Here's how the part is built. I have some questions about the finished solid (model axes, mm). Coordinates: 2 decimals unless noted, no trailing zeros. Write each loop counter-clockwise with the first axis right and the second up, starting at its lowest first coordinate (ties: lowest second). Pieces come first, ordered by that corner, then holes.
Item 1: I'm going to push flat-ended pins straight in: P1, Ø3, axis at x = 7, y = -54.5, coming from the -Z side; P2, Ø7, axis at x = 0, y = -31, coming from the +Z side. Where does each tip first touch, or does it pass through?
Item 2: I want a section at D-D (z = 3.5). Count the separate pieces of the cut face and the enclosed holes in it, and give its area (3 significant figures).
Item 3: I want a section at B-B (y = 46). Please give me the cut outline in (x, z).
Item 4: Please list where these lines run through material, in increasing order: line 1 (Y direction, x = 0, z = 2.8); line 2 (Y direction, x = -20, z = -1.75); line 3 (Y direction, x = -22, z = -1).
Item 5: I want a section at C-C (x = 0). Please give me the cut outline in (y, z), and give its area (3 significant figures).
Item 6: I want a section at A-A (y = -54). Please give me the cut outline in (x, z).
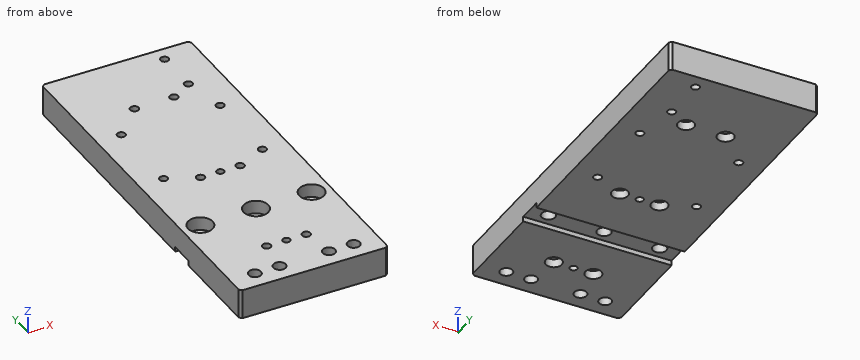
from build123d import *

# Parameters (mm, degrees)
SKETCH1_W                                           = 60
SKETCH1_H                                           = 150
BOSS_EXTRUDE1_DEPTH                                 = 6
M4_TAPPED_HOLE1_D                                   = 3.3
M4_TAPPED_HOLE2_D                                   = 3.3
M4_TAPPED_HOLE2_DEPTH                               = 15.5
M4_TAPPED_HOLE2_TIP                                 = 0.991420021
M6_TAPPED_HOLE2_D                                   = 5
BLIND_PIN_HOLE2_SIZE_MM_D                           = 5
CHAMFER1_SIZE                                       = 1
CBORE_FOR_M3_HEX_SOCKET_HEAD_CAP_SCREW1_D           = 3.4
CBORE_FOR_M3_HEX_SOCKET_HEAD_CAP_SCREW1_CBORE_D     = 6.5
CBORE_FOR_M3_HEX_SOCKET_HEAD_CAP_SCREW1_CBORE_DEPTH = 3.4
LPATTERN1_COUNT                                     = 3
LPATTERN1_PITCH                                     = 50
SKETCH20_R                                          = 1.5
CUT_EXTRUDE1_DEPTH                                  = 82.663945533
SKETCH21_W                                          = 60
SKETCH21_H                                          = 10
CUT_EXTRUDE2_DEPTH                                  = 2
CBORE_FOR_M5_HEX_SOCKET_HEAD_CAP_SCREW1_D           = 5.5
CBORE_FOR_M5_HEX_SOCKET_HEAD_CAP_SCREW1_CBORE_D     = 10
CBORE_FOR_M5_HEX_SOCKET_HEAD_CAP_SCREW1_CBORE_DEPTH = 5.4


with BuildPart() as part:
    # Sketch1 → Boss-Extrude1 (new, symmetric)
    with BuildSketch(Plane.XY):
        Rectangle(SKETCH1_W, SKETCH1_H)
    extrude(amount=BOSS_EXTRUDE1_DEPTH, both=True)

    # M4 Tapped Hole1 (through all)
    with Locations(Plane(origin=(0, 0, -6), x_dir=(-1, 0, 0), z_dir=(0, 0, -1))):
        with Locations((-16.5, 69), (-16.5, 51)):
            Hole(M4_TAPPED_HOLE1_D / 2)

    # M4 Tapped Hole2
    with Locations(Plane(origin=(0, 0, -6), x_dir=(-1, 0, 0), z_dir=(0, 0, -1))):
        with Locations((-20, 33.5), (-20, 1.5), (20, 33.5), (20, 1.5)):
            Hole(M4_TAPPED_HOLE2_D / 2, depth=M4_TAPPED_HOLE2_DEPTH)
            with Locations((0, 0, -(M4_TAPPED_HOLE2_DEPTH + M4_TAPPED_HOLE2_TIP / 2))):  # 118° drill point
                Cone(0, M4_TAPPED_HOLE2_D / 2, M4_TAPPED_HOLE2_TIP, mode=Mode.SUBTRACT)

    # M6 Tapped Hole2 (through all)
    with Locations(Plane(origin=(0, 0, -6), x_dir=(-1, 0, 0), z_dir=(0, 0, -1))):
        with Locations((20, -67.5), (-20, -67.5)):
            Hole(M6_TAPPED_HOLE2_D / 2)

    # Blind Pin Hole2 size mm (through all)
    with Locations(Plane(origin=(0, 0, -6), x_dir=(-1, 0, 0), z_dir=(0, 0, -1))):
        with Locations((10, -67.5), (-10, -67.5)):
            Hole(BLIND_PIN_HOLE2_SIZE_MM_D / 2)

    # Chamfer1
    chamfer1_edges = [part.edges().sort_by_distance(p)[0] for p in [
        (30, -75, 0),
        (-30, -75, 0),
        (-30, 75, 0),
        (30, 75, 0),
    ]]
    chamfer(chamfer1_edges, length=CHAMFER1_SIZE)

    # CBORE for M3 Hex Socket Head Cap Screw1 (through all)
    with Locations(Plane(origin=(0, 0, -6), x_dir=(-1, 0, 0), z_dir=(0, 0, -1))):
        with Locations((8, -54), (-8, -54)):
            cbore_for_m3_hex_socket_head_cap_screw1 = CounterBoreHole(CBORE_FOR_M3_HEX_SOCKET_HEAD_CAP_SCREW1_D / 2, CBORE_FOR_M3_HEX_SOCKET_HEAD_CAP_SCREW1_CBORE_D / 2, CBORE_FOR_M3_HEX_SOCKET_HEAD_CAP_SCREW1_CBORE_DEPTH)

    # LPattern1: CBORE for M3 Hex Socket Head Cap Screw1 ×3
    with Locations(*[(0, i * LPATTERN1_PITCH, 0) for i in range(1, LPATTERN1_COUNT)]):
        add(cbore_for_m3_hex_socket_head_cap_screw1, mode=Mode.SUBTRACT)

    # Sketch20 → Cut-Extrude1 (cut, through all)
    with BuildSketch(Plane(origin=(0, 0, -6), x_dir=(-1, 0, 0), z_dir=(0, 0, -1))):
        with Locations((0, -4)):
            Circle(SKETCH20_R)
        with Locations((0, -54)):
            Circle(SKETCH20_R)
    extrude(amount=-CUT_EXTRUDE1_DEPTH, mode=Mode.SUBTRACT)

    # Sketch21 → Cut-Extrude2 (cut)
    with BuildSketch(Plane(origin=(0, 0, -6), x_dir=(-1, 0, 0), z_dir=(0, 0, -1))):
        with Locations((0, -31)):
            Rectangle(SKETCH21_W, SKETCH21_H)
    extrude(amount=-CUT_EXTRUDE2_DEPTH, mode=Mode.SUBTRACT)

    # CBORE for M5 Hex Socket Head Cap Screw1 (through all)
    with Locations(Plane.XY.offset(6)):
        with Locations((22.5, -31), (0, -31), (-22.5, -31)):
            CounterBoreHole(CBORE_FOR_M5_HEX_SOCKET_HEAD_CAP_SCREW1_D / 2, CBORE_FOR_M5_HEX_SOCKET_HEAD_CAP_SCREW1_CBORE_D / 2, CBORE_FOR_M5_HEX_SOCKET_HEAD_CAP_SCREW1_CBORE_DEPTH)


solid = part.part
Answer:
1. P1: stops at z = -2.6
1. P2: stops at z = 0.6
2. separate pieces: 1
2. enclosed holes: 21
2. area: 8,560 mm2
3. outline: (-30, -6) - (-11.25, -6) - (-11.25, -2.6) - (-9.7, -2.6) - (-9.7, 6) - (-30, 6) - close; (-6.3, -2.6) - (-4.75, -2.6) - (-4.75, -6) - (4.75, -6) - (4.75, -2.6) - (6.3, -2.6) - (6.3, 6) - (-6.3, 6) - close; (9.7, -2.6) - (11.25, -2.6) - (11.25, -6) - (30, -6) - (30, 6) - (9.7, 6) - close
4. line 1: y = -75 to -55.5, -52.5 to -36, -26 to -5.5, -2.5 to 75
4. line 2: y = -75 to -70, -65 to -32.15, -29.85 to -0.15, 3.15 to 31.85, 35.15 to 75
4. line 3: y = -75 to -69, -66 to -33.7, -28.3 to 75
5. outline: (-75, -6) - (-55.5, -6) - (-55.5, 6) - (-75, 6) - close; (-52.5, -6) - (-36, -6) - (-36, -4) - (-33.75, -4) - (-33.75, 0.6) - (-36, 0.6) - (-36, 6) - (-52.5, 6) - close; (-28.25, -4) - (-26, -4) - (-26, -6) - (-5.5, -6) - (-5.5, 6) - (-26, 6) - (-26, 0.6) - (-28.25, 0.6) - close; (-2.5, -6) - (75, -6) - (75, 6) - (-2.5, 6) - close
5. area: 1,630 mm2
6. outline: (-30, -6) - (-11.25, -6) - (-11.25, -2.6) - (-9.7, -2.6) - (-9.7, 6) - (-30, 6) - close; (-6.3, -2.6) - (-4.75, -2.6) - (-4.75, -6) - (-1.5, -6) - (-1.5, 6) - (-6.3, 6) - close; (1.5, -6) - (4.75, -6) - (4.75, -2.6) - (6.3, -2.6) - (6.3, 6) - (1.5, 6) - close; (9.7, -2.6) - (11.25, -2.6) - (11.25, -6) - (30, -6) - (30, 6) - (9.7, 6) - close
